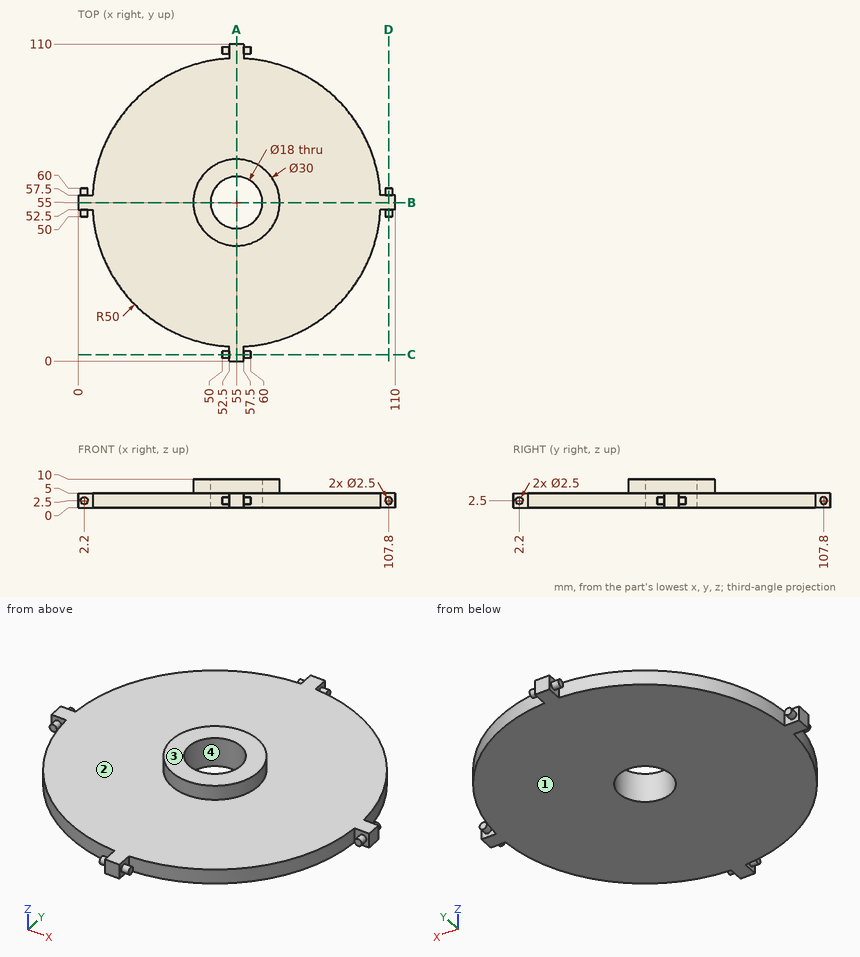
Check sheet for the drawn part. Datum: minimum x, y, z corner. Units: mm. A direction names the side the tool comes from. Round coordinates to 2 decimals unless told otherwise and drop trailing zeros. Order: outer loops, then holes, each group sorted by start corner. A loop starts at its lowest first (then second) coordinate and runs counter-clockwise, first axis right, second up.
(1) Cross-section at A-A, the plane x = 55. Enter the section's corners in (y, z).
(2) Go/stop test with flat-tipped pins: P1, Ø2, axis at y = 98, z = 3, coming from the +X side; P2, Ø1.5, axis at y = 107, z = 3, coming from the -X side; P3, Ø0.8, axis at x = 107.5, z = 2.5, coming from the +Y side; P4, Ø1, axis at y = 27.5, z = 6, coming from the -X side. Record where each tip stops, or that it passes through.
(3) Draft check along X on the marked faces 3 and 4. Enter one of: pulls with the +X half, pulls with the -X half, needs draft (parallel to the pull), parting line crosses it, or undercut.
(4) Access from +Z, -Z, +X, -X, +Y, -Y to the whole of each face (thin tool, end or side, straight path). Record for the marked faces 1 and 2.
(5) Scan lines: probe 1 along Y at (x, z) = (55, 6.75); probe 2 along Z at (x, y) = (24, 63); probe 3 along X at (y, z) = (50, 4.5). Record each from-to range of solid material in increasing order.
(6) Cross-section at C-C, the plane y = 2.2. Enter the section's corners in (x, z), and give its area (3 significant figures).
Check sheet entries:
1. outline: (0, 0) - (46, 0) - (46, 10) - (40, 10) - (40, 5) - (0, 5) - close; (64, 0) - (110, 0) - (110, 5) - (70, 5) - (70, 10) - (64, 10) - close
2. P1: stops at x = 82.13
2. P2: stops at x = 50
2. P3: stops at y = 60
2. P4: passes through
3. face 3: needs draft
3. face 4: undercut
4. face 1: -Z, +X, -X, +Y, -Y
4. face 2: +Z
5. probe 1: y = 40 to 46, 64 to 70
5. probe 2: z = 0 to 5
5. probe 3: x = 5.25 to 47.52, 62.48 to 104.75
6. outline: (50, 1.25) - (52.5, 1.25) - (52.5, 0) - (57.5, 0) - (57.5, 1.25) - (60, 1.25) - (60, 3.75) - (57.5, 3.75) - (57.5, 5) - (52.5, 5) - (52.5, 3.75) - (50, 3.75) - close
6. area: 37.5 mm2
